```python
from build123d import *

# Parameters (mm, degrees)
SKETCH1_W           = 160
SKETCH1_H           = 246
BOSS_EXTRUDE1_DEPTH = 3
SKETCH2_W           = 160
SKETCH2_H           = 3
BOSS_EXTRUDE2_DEPTH = 110


with BuildPart() as part:
    # Sketch1 → Boss-Extrude1 (new body)
    with BuildSketch(Plane.XY):
        Rectangle(SKETCH1_W, SKETCH1_H)
    extrude(amount=BOSS_EXTRUDE1_DEPTH)

    # Sketch2 → Boss-Extrude2 (add)
    with BuildSketch(Plane.XY.offset(3)):
        with Locations((0, 121.5)):
            Rectangle(SKETCH2_W, SKETCH2_H)
        with Locations((0, -121.5)):
            Rectangle(SKETCH2_W, SKETCH2_H)
    extrude(amount=BOSS_EXTRUDE2_DEPTH)


solid = part.part
```
Here's how the part is built. I have some questions about the finished solid (model axes, mm). A direction names the side the tool comes from. Round coordinates to 2 decimals unless told otherwise and drop trailing zeros. Loops run counter-clockwise (first coordinate to the right, second up) from the corner with the lowest first, then second, coordinate; pieces in that order, holes last. Notation, with made-up numbers: (0.25, 41) -> (55.25, 41) arc R17 ccw to (55.25, 68) -> close; hole circle Ø7 at (-17.75, 49.5). An arc over 180 degrees is marked (long way). Answer as CSV lines item,"result". Start each with the question number.
1. I'm going to push flat-ended pins straight in: P1, Ø6, axis at x = -22.5, y = 50.5, coming from the +Z side; P2, Ø10, axis at x = -50.5, y = 48.5, coming from the -Z side. Where does each tip first touch, or does it pass through?
2. I need wall thicknesses on probe 1 along Y at (x, z) = (-20.5, 65); probe 2 along Z at (x, y) = (-56, 65.5). Which ranges of each line are inside material? Lowest first, please. Write a range as from..to.
3. For faces 1 (the face through (80, -1, 2)), 2 (the face through (-1, -120, 57)), which set-ups out of +Z, -Z, +X, -X, +Y, -Y let a thin tool reach every point of the face, with its end or its side?
4. Imagine slicing it at C-C on y = -93. Write out the boundary of the cut face in (x, z).
5. Imagine slicing it at A-A on z = 71. Write out the boundary of the cut face in (x, y).
6. If we mould it in two halves opening along Y, with no side actions, what happens to faces 3 (the face through (-1, -123, 56)), 4 (the face through (-1, 2, 0)), 5 (the face through (-1, 2, 3))? For each: pulls with the +Y half, pulls with the -Y half, needs draft (parallel to the pull), parting line crosses it, or undercut.
7. Imagine slicing it at B-B on x = 35.5. Write out the boundary of the cut face in (y, z).
Solution:
1,P1,"z = 3"
1,P2,"z = 0"
2,probe 1,"-123..-120, 120..123"
2,probe 2,"0..3"
3,face 1,"+Z, -Z, +X, +Y, -Y"
3,face 2,"+Z, +X, -X"
4,outline,"(-80, 0) -> (80, 0) -> (80, 3) -> (-80, 3) -> close"
5,outline,"(-80, -123) -> (80, -123) -> (80, -120) -> (-80, -120) -> close; (-80, 120) -> (80, 120) -> (80, 123) -> (-80, 123) -> close"
6,face 3,"pulls with the -Y half"
6,face 4,"needs draft"
6,face 5,"undercut"
7,outline,"(-123, 0) -> (123, 0) -> (123, 113) -> (120, 113) -> (120, 3) -> (-120, 3) -> (-120, 113) -> (-123, 113) -> close"
